Geometry check sheet. Reference: the model listing, model coordinates, mm. A direction names the side the tool comes from. Round coordinates to 2 decimals unless told otherwise and drop trailing zeros. Loops run counter-clockwise (first coordinate to the right, second up) from the corner with the lowest first, then second, coordinate; pieces in that order, holes last. Notation, with made-up numbers: (23.5, -24) - (48.5, -24) arc R9 ccw to (48.5, -15) - close; hole circle Ø1 at (53.5, -5). An arc over 180 degrees is marked (long way). Answer in a Markdown table with one row per item. Add a question column.
```python
from build123d import *

# Parameters (mm, degrees)
SKETCH1_R          = 6.9175
EXTRUDE1_DEPTH     = 16.4
SKETCH2_OUTSIDE_W  = 34.032
SKETCH2_OUTSIDE_H  = 37.744
SKETCH2_OUTSIDE_R  = 11.25
CUT_EXTRUDE2_DEPTH = 0.8
SKETCH3_OUTSIDE_W  = 122.7
SKETCH3_OUTSIDE_H  = 126.412
SKETCH3_OUTSIDE_R  = 12
CUT_EXTRUDE3_DEPTH = 25.595934623
CUT_EXTRUDE3_DRAFT = -60
CHAMFER1_SIZE      = 0.82


with BuildPart() as part:
    # Sketch1 → Extrude1 (new body)
    with BuildSketch(Plane.XY):
        Polygon((0, 13.856406461), (-12, 6.92820323), (-12, -6.92820323), (0, -13.856406461), (12, -6.92820323), (12, 6.92820323), align=None)
        Circle(SKETCH1_R, mode=Mode.SUBTRACT)
    extrude(amount=EXTRUDE1_DEPTH)

    # Sketch2 outside → Cut-Extrude2 (cut)
    with BuildSketch(Plane.XY):
        Rectangle(SKETCH2_OUTSIDE_W, SKETCH2_OUTSIDE_H)
        Circle(SKETCH2_OUTSIDE_R, mode=Mode.SUBTRACT)
    extrude(amount=CUT_EXTRUDE2_DEPTH, mode=Mode.SUBTRACT)


with BuildPart() as cut_extrude3_tool:
    # Sketch3 outside → Cut-Extrude3 (with draft: the straight prism first)
    with BuildSketch(Plane.XY.offset(16.4)):
        Rectangle(SKETCH3_OUTSIDE_W, SKETCH3_OUTSIDE_H)
        Circle(SKETCH3_OUTSIDE_R, mode=Mode.SUBTRACT)
    extrude(amount=-CUT_EXTRUDE3_DEPTH)
    # Cut-Extrude3: the draft: its side faces are tilted about the plane it starts from
    cut_extrude3_sides = [cut_extrude3_tool.faces().sort_by_distance(p)[0] for p in [
        (0, -63.206, 3.602032688),
        (61.35, 0, 3.602032688),
        (0, 63.206, 3.602032688),
        (-61.35, 0, 3.602032688),
        (-12, 0, 3.602032688),
    ]]
    draft(cut_extrude3_sides, Plane.XY.offset(16.4), CUT_EXTRUDE3_DRAFT)


with BuildPart() as part_1:
    add(part.part)

    # Cut-Extrude3: cut by cut_extrude3_tool
    add(cut_extrude3_tool.part, mode=Mode.SUBTRACT)

    # Chamfer1
    chamfer1_edges = [part_1.edges().sort_by_distance(p)[0] for p in [
        (-6.9175, 0, 0),
        (-6.9175, 0, 16.4),
    ]]
    chamfer(chamfer1_edges, length=CHAMFER1_SIZE)


solid = part_1.part
```
Q1. Release check for a two-part mould opening along Y. For faces 1 (the cylindrical face through (-6.91, 0.3, 8.1)), 2 (the flat face through (-0.1, 11.4, 0.8)), 3 (the flat face through (6.084, 10.344, 8.491)) record: +Y half, -Y half, draft (parallel to the pull), parting line (faces both ways), or undercut.
Q2. Depth check by flat-ended pin: P1, Ø4, axis at x = -1, z = 4, coming from the -Y side. Enter the tip coordinate at first touch or a pass-through.
Q3. Set-up check for faces 4 (the cylindrical face through (5.19, -9.98, 0.39)), 5 (the flat face through (0, -8, 16.4)): record each of +Z, -Z, +X, -X, +Y, -Y from which the full face is reachable in a straight line by a thin tool's end or side.
Q4. Cross-section at A-A, the plane z = 2. Enter the section's corners in (x, y) (1 decimal), plus the area to 4 significant figures.
Q5. Scan lines: line 1 (Z direction, x = 0, y = -12); line 2 (X direction, y = 5.5, z = 13.75); line 3 (X direction, y = 1.75, z = 14.25). Record each from-to range of solid material in increasing order. Write a range as from..to.
Check sheet entries:
| question | item | result |
|---|---|---|
| 1 | face 1 | undercut |
| 1 | face 2 | draft |
| 1 | face 3 | +Y half |
| 2 | P1 | y = -13.86 |
| 3 | face 4 | -Z |
| 3 | face 5 | +Z, +X, -X, +Y, -Y |
| 4 | outline | (-12, -6.9) - (0, -13.9) - (12, -6.9) - (12, 6.9) - (0, 13.9) - (-12, 6.9) - close; hole circle Ø13.8 at (0, 0) |
| 4 | area | 348.5 mm² |
| 5 | line 1 | 0.8..16.4 |
| 5 | line 2 | -12..-4.2, 4.2..12 |
| 5 | line 3 | -12..-6.69, 6.69..12 |
